from build123d import *

# Parameters (mm, degrees)
BASE_PLATE_SKETCH_R      = 5
BASE_PLATE_DEPTH         = 10
BASE_PLATE_2_DEPTH       = 10
HOUSING_BLOCK_DEPTH      = 66
ARCH_OPENING_CUT_DEPTH   = 10
HOUSING_START            = -10
HOUSING_RELIEF_CUT_DEPTH = 10
PIVOT_BARREL_SKETCH_R    = 15
PIVOT_BARREL_SKETCH_R_2  = 8
PIVOT_BARREL_DEPTH       = 44
PIVOT_BORE_SKETCH_R      = 8
PIVOT_BORE_16_DEPTH      = 44
SIDE_START               = 25.5
SIDE_BOSS_A_SKETCH_R     = 15
SIDE_BOSS_A_SKETCH_R_2   = 8
SIDE_BOSS_A_DEPTH        = 25.5
SIDE_BOSS_B_SKETCH_R     = 15
SIDE_BOSS_B_SKETCH_R_2   = 8
SIDE_BOSS_B_DEPTH        = 25.5
SIDE_WEB_B_SKETCH_W      = 8
SIDE_WEB_B_SKETCH_H      = 17
SIDE_WEB_B_DEPTH         = 25.5
SIDE_WEB_A_SKETCH_W      = 8
SIDE_WEB_A_SKETCH_H      = 17
SIDE_WEB_A_DEPTH         = 25.5
GUSSET_RIB_DEPTH         = 4


with BuildPart() as part:
    # Base Plate Sketch → Base Plate (new body)
    with BuildSketch(Plane(origin=(0, 0, 0), x_dir=(1, 0, 0), z_dir=(0, 1, 0))):
        with BuildLine():
            Line((-55.5, 33), (-22, 33))
            Line((-22, 33), (-22, -33))
            Line((-22, -33), (-55.5, -33))
            ThreePointArc((-55.5, -33), (-63.985281374, -29.485281374), (-67.5, -21))
            Line((-67.5, -21), (-67.5, 21))
            ThreePointArc((-67.5, 21), (-63.985281374, 29.485281374), (-55.5, 33))
        make_face()
        with Locations(Location((-55.5, 21, 0), (0, 0, 270))):
            Circle(BASE_PLATE_SKETCH_R, mode=Mode.SUBTRACT)
        with Locations(Location((-55.5, -21, 0), (0, 0, 270))):
            Circle(BASE_PLATE_SKETCH_R, mode=Mode.SUBTRACT)
    extrude(amount=BASE_PLATE_DEPTH)



with BuildPart() as body_2:
    # Base Plate Sketch → Base Plate 2 (new body)
    with BuildSketch(Plane(origin=(0, 0, 0), x_dir=(1, 0, 0), z_dir=(0, 1, 0))):
        with BuildLine():
            Line((67.5, 21), (67.5, -21))
            ThreePointArc((67.5, -21), (63.985281374, -29.485281374), (55.5, -33))
            Line((55.5, -33), (22, -33))
            Line((22, -33), (22, 33))
            Line((22, 33), (55.5, 33))
            ThreePointArc((55.5, 33), (63.985281374, 29.485281374), (67.5, 21))
        make_face()
        with Locations(Location((55.5, 21, 0), (0, 0, 270))):
            Circle(BASE_PLATE_SKETCH_R, mode=Mode.SUBTRACT)
        with Locations(Location((55.5, -21, 0), (0, 0, 270))):
            Circle(BASE_PLATE_SKETCH_R, mode=Mode.SUBTRACT)
    extrude(amount=BASE_PLATE_2_DEPTH)


with BuildPart() as part_1:
    add(part.part)

    add(body_2.part)  # Housing Block merges body 2
    # Housing Block Sketch → Housing Block (add)
    with BuildSketch(Plane.XY.offset(33)):
        with BuildLine():
            Line((-22, 54), (-22, 10))
            Line((-22, 10), (-22, 0))
            Line((-22, 0), (-13, 0))
            Line((-13, 0), (-13, 54))
            ThreePointArc((-13, 54), (0, 67), (13, 54))
            Line((13, 54), (13, 0))
            Line((13, 0), (22, 0))
            Line((22, 0), (22, 54))
            ThreePointArc((22, 54), (0, 76), (-22, 54))
        make_face()
    extrude(amount=-HOUSING_BLOCK_DEPTH)

    # Arch Opening Sketch → Arch Opening Cut (cut)
    with BuildSketch(Plane.XY.offset(33)):
        with BuildLine():
            Line((13, 54), (13, 35))
            Line((13, 35), (22, 35))
            Line((22, 35), (22, 54))
            ThreePointArc((22, 54), (0, 76), (-22, 54))
            Line((-22, 54), (-22, 35))
            Line((-22, 35), (-13, 35))
            Line((-13, 35), (-13, 54))
            ThreePointArc((-13, 54), (0, 67), (13, 54))
        make_face()
    extrude(amount=-ARCH_OPENING_CUT_DEPTH, mode=Mode.SUBTRACT)

    # Housing Relief Sketch → Housing Relief Cut (cut)
    with BuildSketch(Plane(origin=(0, 0, -33), x_dir=(-1, 0, 0), z_dir=(0, 0, -1)).offset(HOUSING_START)):
        with BuildLine():
            Line((-13, 35), (-22, 35))
            Line((-22, 35), (-22, 54))
            ThreePointArc((-22, 54), (0, 76), (22, 54))
            Line((22, 54), (22, 35))
            Line((22, 35), (13, 35))
            Line((13, 35), (13, 54))
            ThreePointArc((13, 54), (0, 67), (-13, 54))
            Line((-13, 54), (-13, 35))
        make_face()
    extrude(amount=HOUSING_RELIEF_CUT_DEPTH, mode=Mode.SUBTRACT)

    # Pivot Barrel Sketch → Pivot Barrel (add)
    with BuildSketch(Plane.ZY.offset(22)):
        with Locations((0, 35)):
            Circle(PIVOT_BARREL_SKETCH_R)
        with Locations((0, 35)):
            Circle(PIVOT_BARREL_SKETCH_R_2, mode=Mode.SUBTRACT)
    extrude(amount=-PIVOT_BARREL_DEPTH)

    # Pivot Bore Sketch → Pivot Bore Ø16 (cut)
    with BuildSketch(Plane.ZY.offset(22)):
        with Locations((0, 35)):
            Circle(PIVOT_BORE_SKETCH_R)
    extrude(amount=-PIVOT_BORE_16_DEPTH, mode=Mode.SUBTRACT)

    # Side Boss A Sketch → Side Boss A (add)
    with BuildSketch(Plane.ZY.offset(22).offset(SIDE_START)):
        with Locations((0, 35)):
            Circle(SIDE_BOSS_A_SKETCH_R)
        with Locations((0, 35)):
            Circle(SIDE_BOSS_A_SKETCH_R_2, mode=Mode.SUBTRACT)
    extrude(amount=-SIDE_BOSS_A_DEPTH)

    # Side Boss B Sketch → Side Boss B (add)
    with BuildSketch(Plane(origin=(22, 0, 0), x_dir=(0, 0, -1), z_dir=(1, 0, 0))):
        with Locations(Location((0, 35, 0), (0, 0, 180))):
            Circle(SIDE_BOSS_B_SKETCH_R)
        with Locations(Location((0, 35, 0), (0, 0, 180))):
            Circle(SIDE_BOSS_B_SKETCH_R_2, mode=Mode.SUBTRACT)
    extrude(amount=SIDE_BOSS_B_DEPTH)

    # Side Web B Sketch → Side Web B (add)
    with BuildSketch(Plane(origin=(47.5, 0, 0), x_dir=(0, 0, -1), z_dir=(1, 0, 0))):
        with Locations((0, 18.5)):
            Rectangle(SIDE_WEB_B_SKETCH_W, SIDE_WEB_B_SKETCH_H)
    extrude(amount=-SIDE_WEB_B_DEPTH)

    # Side Web A Sketch → Side Web A (add)
    with BuildSketch(Plane.ZY.offset(47.5)):
        with Locations((0, 18.5)):
            Rectangle(SIDE_WEB_A_SKETCH_W, SIDE_WEB_A_SKETCH_H)
    extrude(amount=-SIDE_WEB_A_DEPTH)

    # Gusset Rib Sketch → Gusset Rib (add, symmetric)
    with BuildSketch(Plane.XY):
        with BuildLine():
            Line((-11.755648115, 72.595825806), (-47.5, 50))
            Line((-47.5, 50), (-47.5, 44))
            Line((-47.5, 44), (-22, 44))
            Line((-22, 44), (-22, 54))
            ThreePointArc((-22, 54), (-19.269461053, 64.615454335), (-11.755648115, 72.595825806))
        make_face()
        with BuildLine():
            Line((47.5, 50), (12.615670058, 72.023453304))
            ThreePointArc((12.615670058, 72.023453304), (19.513389522, 64.16009987), (22, 54))
            Line((22, 54), (22, 44))
            Line((22, 44), (47.5, 44))
            Line((47.5, 44), (47.5, 50))
        make_face()
    extrude(amount=GUSSET_RIB_DEPTH, both=True)


solid = part_1.part
Verification items for the finished model (mm, model axes). A direction names the side the tool comes from. Give positions to 0.01 mm unless a question says otherwise; leave off trailing zeros. Loops run counter-clockwise (first coordinate to the right, second up) from the corner with the lowest first, then second, coordinate; pieces in that order, holes last. Notation, with made-up numbers: (-22, 19) - (6, 19) arc R21 cw to (6, 53) - close; hole circle Ø9 at (-24.5, -6). An arc over 180 degrees is marked (long way). Write item = value, one per line. Start each with the question number.
Q1. Mould release check, pull along Z, two halves, no side actions. Record for faces 1 (the face through (35, 35, -15)), 2 (the face through (-18, 35, 28)), 3 (the face through (-50.543, 4.93, -21.651)): released by +Z, released by -Z, zero draft, split by the parting line, or undercut.
Q2. Cross-section at A-A, the plane x = 0. Enter the section's corners in (y, z).
Q3. Thickness scan on line 1 (X direction, y = 6, z = -21); line 2 (X direction, y = 6, z = -13); line 3 (Z direction, x = -55, y = 4). Record the ranges inside material, lowest first.
Q4. Cross-section at C-C, the plane y = 13.5. Enter the section's corners in (x, z), and give its area (3 significant figures).
Q5. Cross-section at B-B, the plane z = -12. Enter the section's corners in (x, y), and give its area (3 significant figures).
Q6. Cross-section at D-D, the plane z = 6. Enter the section's corners in (x, y).
Q7. Tool access check on faces 4 (the face through (-10, 65, -23)), 5 (the face through (-10, 65, 23)), 6 (the face through (35, 15, 4)), 7 (the face through (50, 10, 0)). Record the directions out of +Z, -Z, +X, -X, +Y, -Y that give a thin tool (end or side, any length) a straight path to the whole face; none if there is none.
Q8. Depth check by flat-ended pin: P1, Ø5.5, axis at x = 39, y = 15, coming from the -Z side; P2, Ø5.5, axis at x = 32, y = 15, coming from the +Z side; P3, Ø3, axis at y = 12.5, z = -1, coming from the +X side; P4, Ø8, axis at x = 55.5, z = -21, coming from the +Y side. Enter the tip coordinate at first touch or a pass-through.
Answer key:
q1.face_1 = released by -Z
q1.face_2 = zero draft
q1.face_3 = undercut
q2.outline = circle Ø30 at (35, 0); (67, -23) - (76, -23) - (76, 23) - (67, 23) - close; hole circle Ø16 at (35, 0)
q3.line_1 = -67.5 to -60.5, -50.5 to -13, 13 to 50.5, 60.5 to 67.5
q3.line_2 = -67.5 to -13, 13 to 67.5
q3.line_3 = -33 to -25.97, -16.03 to 16.03, 25.97 to 33
q4.outline = (-47.5, -4) - (-22, -4) - (-22, -33) - (-13, -33) - (-13, 33) - (-22, 33) - (-22, 4) - (-47.5, 4) - close; (13, -33) - (22, -33) - (22, -4) - (47.5, -4) - (47.5, 4) - (22, 4) - (22, 33) - (13, 33) - close
q4.area = 1,600 mm^2
q5.outline = (-67.5, 0) - (-13, 0) - (-13, 26) - (13, 26) - (13, 0) - (67.5, 0) - (67.5, 10) - (22, 10) - (22, 26) - (47.5, 26) - (47.5, 44) - (22, 44) - (22, 54) arc R22 ccw to (-22, 54) - (-22, 44) - (-47.5, 44) - (-47.5, 26) - (-22, 26) - (-22, 10) - (-67.5, 10) - close; hole (-13, 44) - (13, 44) - (13, 54) arc R13 ccw to (-13, 54) - close
q5.area = 3,760 mm^2
q6.outline = (-67.5, 0) - (-13, 0) - (-13, 21.25) - (13, 21.25) - (13, 0) - (67.5, 0) - (67.5, 10) - (22, 10) - (22, 21.25) - (47.5, 21.25) - (47.5, 29.71) - (-47.5, 29.71) - (-47.5, 21.25) - (-22, 21.25) - (-22, 10) - (-67.5, 10) - close; (-47.5, 40.29) - (47.5, 40.29) - (47.5, 48.75) - (22, 48.75) - (22, 54) arc R22 ccw to (-22, 54) - (-22, 48.75) - (-47.5, 48.75) - close; hole (-13, 48.75) - (13, 48.75) - (13, 54) arc R13 ccw to (-13, 54) - close
q7.face_4 = -Z, +X, -X, +Y
q7.face_5 = +Z, +X, -X, +Y
q7.face_6 = +Z, +X
q7.face_7 = +X
q8.P1 = -4
q8.P2 = 4
q8.P3 = 47.5
q8.P4 = through
